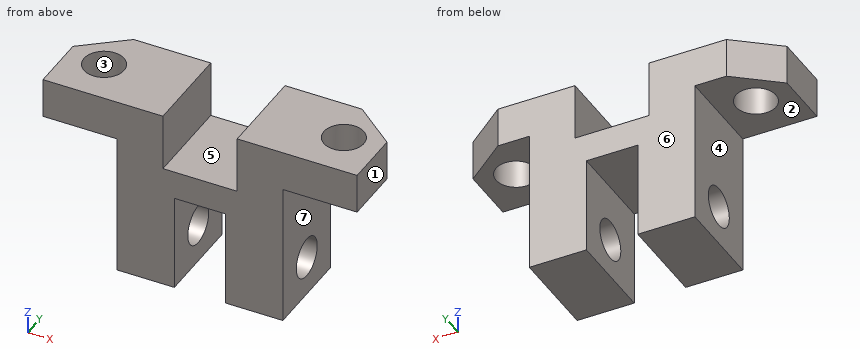
```python
from build123d import *

# Parameters (mm, degrees)
BASE_BLOCK_PROFILE_W        = 55
BASE_BLOCK_PROFILE_H        = 16
BASE_BLOCK_DEPTH            = 32
CENTRE_NOTCH_DEPTH          = 46.124826869
CENTRE_NOTCH_DEPTH_BACK     = 46.124826869
CENTRE_NOTCH_PROFILE_W      = 13
CENTRE_NOTCH_PROFILE_H      = 25
SIDE_STEP_CUT_DEPTH         = 46.124826869
SIDE_STEP_CUT_DEPTH_BACK    = 46.124826869
SIDE_STEP_CUT_PROFILE_W     = 13
SIDE_STEP_CUT_PROFILE_H     = 10
CORNER_BEVEL_CUT_DEPTH      = 46.124826869
CORNER_BEVEL_CUT_DEPTH_BACK = 46.124826869
CORNER_BEVEL_PROFILE_W      = 9
CORNER_BEVEL_PROFILE_H      = 17
LUG_SLOT_CUT_DEPTH          = 39.016443811
LUG_SLOT_CUT_DEPTH_BACK     = 39.016443811
LUG_HOLES_7_DEPTH           = 39.016443811
LUG_HOLES_7_DEPTH_BACK      = 39.016443811
LUG_HOLES_7_SKETCH_R        = 3.5
CROSS_HOLE_7_DEPTH          = 54.404119691
CROSS_HOLE_7_DEPTH_BACK     = 54.404119691
CROSS_HOLE_7_SKETCH_R       = 3.5


with BuildPart() as part:
    # Base Block Profile → Base Block (new body)
    with BuildSketch(Plane.XY):
        Rectangle(BASE_BLOCK_PROFILE_W, BASE_BLOCK_PROFILE_H)
    extrude(amount=BASE_BLOCK_DEPTH)

    # Centre Notch Profile → Centre Notch (cut, two sides: drawn at the far end of the back side and taken through both)
    with BuildSketch(Plane(origin=(0, 8, 0), x_dir=(1, 0, 0), z_dir=(0, 1, 0)).offset(-CENTRE_NOTCH_DEPTH_BACK)):
        with Locations((-21, -12.5)):
            Rectangle(CENTRE_NOTCH_PROFILE_W, CENTRE_NOTCH_PROFILE_H)
        with Locations((21, -12.5)):
            Rectangle(CENTRE_NOTCH_PROFILE_W, CENTRE_NOTCH_PROFILE_H)
    extrude(amount=CENTRE_NOTCH_DEPTH + CENTRE_NOTCH_DEPTH_BACK, mode=Mode.SUBTRACT)

    # Side Step Cut Profile → Side Step Cut (cut, two sides: drawn at the far end of the back side and taken through both)
    with BuildSketch(Plane(origin=(0, 8, 0), x_dir=(1, 0, 0), z_dir=(0, 1, 0)).offset(-SIDE_STEP_CUT_DEPTH_BACK)):
        with Locations((0, -27)):
            Rectangle(SIDE_STEP_CUT_PROFILE_W, SIDE_STEP_CUT_PROFILE_H)
    extrude(amount=SIDE_STEP_CUT_DEPTH + SIDE_STEP_CUT_DEPTH_BACK, mode=Mode.SUBTRACT)

    # Corner Bevel Profile → Corner Bevel Cut (cut, two sides: drawn at the far end of the back side and taken through both)
    with BuildSketch(Plane(origin=(0, 8, 0), x_dir=(1, 0, 0), z_dir=(0, 1, 0)).offset(-CORNER_BEVEL_CUT_DEPTH_BACK)):
        with Locations((0, -8.5)):
            Rectangle(CORNER_BEVEL_PROFILE_W, CORNER_BEVEL_PROFILE_H)
    extrude(amount=CORNER_BEVEL_CUT_DEPTH + CORNER_BEVEL_CUT_DEPTH_BACK, mode=Mode.SUBTRACT)

    # Lug Slot Profile → Lug Slot Cut (cut, two sides: drawn at the far end of the back side and taken through both)
    with BuildSketch(Plane(origin=(0, 0, 25), x_dir=(-1, 0, 0), z_dir=(0, 0, -1)).offset(-LUG_SLOT_CUT_DEPTH_BACK)):
        Polygon((-27.5, 8), (-20, 8), (-27.5, 2), align=None)
        Polygon((20, 8), (27.5, 2), (27.5, 8), align=None)
    extrude(amount=LUG_SLOT_CUT_DEPTH + LUG_SLOT_CUT_DEPTH_BACK, mode=Mode.SUBTRACT)

    # Lug Holes _7 Sketch → Lug Holes _7 (cut, two sides: drawn at the far end of the back side and taken through both)
    with BuildSketch(Plane(origin=(0, 0, 25), x_dir=(-1, 0, 0), z_dir=(0, 0, -1)).offset(-LUG_HOLES_7_DEPTH_BACK)):
        with BuildLine():
            ThreePointArc((24.5, 0), (21, 3.5), (17.5, 0))
            Line((17.5, 0), (24.5, 0))
        make_face()
        with BuildLine():
            Line((24.5, 0), (17.5, 0))
            ThreePointArc((17.5, 0), (21, -3.5), (24.5, 0))
        make_face()
        with Locations((-21, 0)):
            Circle(LUG_HOLES_7_SKETCH_R)
    extrude(amount=LUG_HOLES_7_DEPTH + LUG_HOLES_7_DEPTH_BACK, mode=Mode.SUBTRACT)

    # Cross Hole _7 Sketch → Cross Hole _7 (cut, two sides: drawn at the far end of the back side and taken through both)
    with BuildSketch(Plane(origin=(14.5, 0, 0), x_dir=(0, 0, -1), z_dir=(1, 0, 0)).offset(-CROSS_HOLE_7_DEPTH_BACK)):
        with Locations((-7, 0)):
            Circle(CROSS_HOLE_7_SKETCH_R)
    extrude(amount=CROSS_HOLE_7_DEPTH + CROSS_HOLE_7_DEPTH_BACK, mode=Mode.SUBTRACT)


solid = part.part
```
Build history of the part. All positions in model axes, mm. Face numbers are marked on the shaded views. A direction names the side the tool comes from. Round coordinates to 2 decimals unless told otherwise and drop trailing zeros. Write each loop counter-clockwise with the first axis right and the second up, starting at its lowest first coordinate (ties: lowest second). Pieces come first, ordered by that corner, then holes. Notation, with made-up numbers: (-3.75, 60) -> (11.25, 60) arc R26 ccw to (11.25, 95) -> close; hole circle Ø3 at (-7, 49). An arc over 180 degrees is marked (long way). Put each result on its own line as item: value.
Item 1: Tool access for the marked faces 4, 5, 6 and 7: list every direction of +Z, -Z, +X, -X, +Y, -Y with a clear straight run to the whole face (end or side of a thin tool).
Here are the results:
face 4: -Z, -X, +Y, -Y
face 5: +Z, +Y, -Y
face 6: +Z, -Z, +X, -X, +Y
face 7: -Z, +X, +Y, -Y
Item 2: Slice it at C-C, the plane z = 7. Give the cut face in (x, y), plus the area to 3 significant figures.
Here are the results:
outline: (-14.5, -8) -> (-4.5, -8) -> (-4.5, -3.5) -> (-14.5, -3.5) -> close; (-14.5, 3.5) -> (-4.5, 3.5) -> (-4.5, 8) -> (-14.5, 8) -> close; (4.5, -8) -> (14.5, -8) -> (14.5, -3.5) -> (4.5, -3.5) -> close; (4.5, 3.5) -> (14.5, 3.5) -> (14.5, 8) -> (4.5, 8) -> close
area: 180 mm^2
Item 3: Slice it at B-B, the plane y = 0. Count the separate pieces of the cut face and the enclosed holes in it, plus the area to 3 significant figures.
Here are the results:
separate pieces: 5
enclosed holes: 0
area: 589 mm^2
Item 4: Flat gauge pins, fed straight in: P1, Ø8, axis at y = 1, z = 6.5, coming from the +X side; P2, Ø7, axis at x = 0.5, y = -2, coming from the -Z side; P3, Ø5.5, axis at y = 0, z = 7, coming from the +X side; P4, Ø6.5, axis at x = -1.5, y = 1, coming from the +Z side. Where does each tip first touch, or does it go through?
Here are the results:
P1: stops at x = 14.5
P2: stops at z = 17
P3: passes through
P4: stops at z = 22
Item 5: Slice it at A-A, the plane z = 26. Give the cut face in (x, y), plus the area to 3 significant figures.
Here are the results:
outline: (-27.5, -8) -> (-6.5, -8) -> (-6.5, 8) -> (-20, 8) -> (-27.5, 2) -> close; (6.5, -8) -> (27.5, -8) -> (27.5, 2) -> (20, 8) -> (6.5, 8) -> close; hole circle Ø7 at (-21, 0); hole circle Ø7 at (21, 0)
area: 550 mm^2
Item 6: Wall check: probe 1 along Y at (x, z) = (-6.5, 7); probe 2 along X at (y, z) = (6.5, 14); probe 3 along Z at (x, y) = (-8, 0). Give the ranges that are in metal, low to high. Write a range as from..to.
Here are the results:
probe 1: y = -8..-3.5, 3.5..8
probe 2: x = -14.5..-4.5, 4.5..14.5
probe 3: z = 0..3.5, 10.5..32
Item 7: Two-plate mould, pull along X, no slides. Class the marked faces 1, 2 and 3: pulls with the +X half, pulls with the -X half, needs draft (parallel to the pull), parting line crosses it, or undercut.
Here are the results:
face 1: pulls with the +X half
face 2: needs draft
face 3: undercut
Item 8: Slice it at D-D, the plane x = 21. Give the cut face in (y, z), plus the area to 3 significant figures.
Here are the results:
outline: (-8, 25) -> (-3.5, 25) -> (-3.5, 32) -> (-8, 32) -> close; (3.5, 25) -> (7.2, 25) -> (7.2, 32) -> (3.5, 32) -> close
area: 57.4 mm^2
